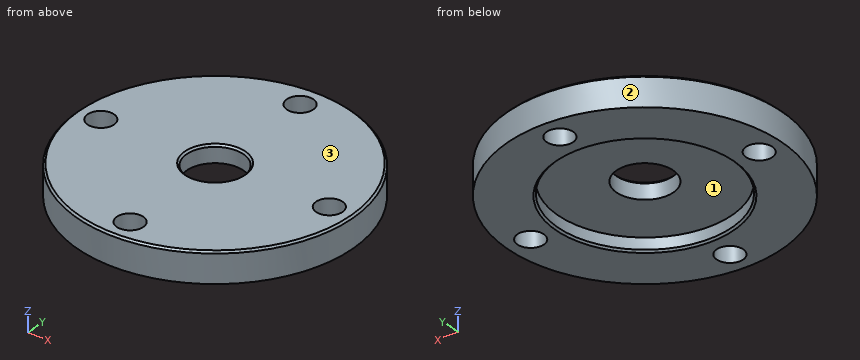
from build123d import *

# Parameters (mm, degrees)
SKETCH_1_R          = 72.5
EXTRUDE_1_DEPTH     = 16
SKETCH_2_R          = 7
CUT_EXTRUDE_1_DEPTH = 104.771383339
SKETCH_3_R          = 46
CUT_EXTRUDE_2_DEPTH = 7
SKETCH_4_R          = 15
CUT_EXTRUDE_3_DEPTH = 104.771383339
CHAMFER_1_SIZE      = 1


with BuildPart() as part:
    # 草图1 → 凸台-拉伸1 (new body)
    with BuildSketch(Plane.XY):
        Circle(SKETCH_1_R)
    extrude(amount=EXTRUDE_1_DEPTH)

    # 草图2 → 切除-拉伸1 (cut, through all)
    with BuildSketch(Plane.XY.offset(16)):
        with Locations((0, 60)):
            Circle(SKETCH_2_R)
        with Locations((60, 0)):
            Circle(SKETCH_2_R)
        with Locations((0, -60)):
            Circle(SKETCH_2_R)
        with Locations((-60, 0)):
            Circle(SKETCH_2_R)
    extrude(amount=-CUT_EXTRUDE_1_DEPTH, mode=Mode.SUBTRACT)

    # 草图3 → 切除-拉伸2 (cut)
    with BuildSketch(Plane(origin=(0, 0, 0), x_dir=(-1, 0, 0), z_dir=(0, 0, -1))):
        Circle(SKETCH_3_R)
    extrude(amount=-CUT_EXTRUDE_2_DEPTH, mode=Mode.SUBTRACT)

    # 草图4 → 切除-拉伸3 (cut, through all)
    with BuildSketch(Plane.XY.offset(16)):
        Circle(SKETCH_4_R)
    extrude(amount=-CUT_EXTRUDE_3_DEPTH, mode=Mode.SUBTRACT)

    # 倒角1
    chamfer_1_edges = [part.edges().sort_by_distance(p)[0] for p in [
        (46, 0, 0),
        (-15, 0, 16),
        (-72.5, 0, 16),
    ]]
    chamfer(chamfer_1_edges, length=CHAMFER_1_SIZE)


solid = part.part
Verification items for the finished model (mm, model axes). Face numbers are marked on the shaded views. Coordinates: 2 decimals unless noted, no trailing zeros. Order: outer loops, then holes, each group sorted by start corner. A loop starts at its lowest first (then second) coordinate and runs counter-clockwise, first axis right, second up. Notation, with made-up numbers: (42, 22) -> (97, 22) arc R13 ccw to (97, 40) -> close; hole circle Ø5 at (58.25, 54). An arc over 180 degrees is marked (long way). Put each result on its own line as item: value. Start each with the question number.
1. Material ranges on L1, parallel to Z at x = 6, y = -34.5; L2, parallel to X at y = 18.5, z = 4.25; L3, parallel to X at y = 64, z = 9.75, recorded low to high. Write a range as [from, to].
2. Cross-section at A-A, the plane x = 0. Record the boundary of the cut face in (y, z), then the cut area to 3 significant figures.
3. Go/stop test with flat-tipped pins: pin 1 Ø6 at (y, z) = (39.5, 2) entering from -X; pin 2 Ø2 at (y, z) = (27, 10) entering from +X; pin 3 Ø11 at (x, y) = (-60, 0) entering from +Z; pin 4 Ø8 at (x, z) = (9.5, 7) entering from +Y. Record where each tip stops, or that it passes through.
4. Cross-section at C-C, the plane z = 4.75. Record the boundary of the cut face in (x, y), then the cut area to 3 significant figures.
5. Mould release check, pull along Y, two halves, no side actions. Record for the marked faces 1, 2 and 3: released by +Y, released by -Y, zero draft, split by the parting line, or undercut.
Computed:
1. L1: [7, 16]
1. L2: [-70.1, -42.12], [42.12, 70.1]
1. L3: [-34.06, -5.74], [5.74, 34.06]
2. outline: (-72.5, 0) -> (-67, 0) -> (-67, 16) -> (-71.5, 16) -> (-72.5, 15) -> close; (-53, 0) -> (-47, 0) -> (-46, 1) -> (-46, 7) -> (-15, 7) -> (-15, 15) -> (-16, 16) -> (-53, 16) -> close; (15, 7) -> (46, 7) -> (46, 1) -> (47, 0) -> (53, 0) -> (53, 16) -> (16, 16) -> (15, 15) -> close; (67, 0) -> (72.5, 0) -> (72.5, 15) -> (71.5, 16) -> (67, 16) -> close
2. area: 955 mm2
3. pin 1: x = -62.64
3. pin 2: x = 67.68
3. pin 3: through
3. pin 4: y = 72.29
4. outline: circle Ø145 at (0, 0); hole circle Ø14 at (-60, 0); hole circle Ø92 at (0, 0); hole circle Ø14 at (0, -60); hole circle Ø14 at (0, 60); hole circle Ø14 at (60, 0)
4. area: 9,250 mm2
5. face 1: undercut
5. face 2: split by the parting line
5. face 3: zero draft
